Could you check a few things on this model? Use its own coordinates, in mm. Round coordinates to 2 decimals unless told otherwise and drop trailing zeros. Order: outer loops, then holes, each group sorted by start corner. A loop starts at its lowest first (then second) coordinate and runs counter-clockwise, first axis right, second up. Notation, with made-up numbers: (43.25, 69.25) -> (85.25, 69.25) arc R26 ccw to (85.25, 94.25) -> close; hole circle Ø4 at (-14, 16). An arc over 180 degrees is marked (long way). One line per question, with ' | ' between items.
```python
from build123d import *

# Parameters (mm, degrees)
SKETCH1_R           = 12.75
BOSS_EXTRUDE1_DEPTH = 12


with BuildPart() as part:
    # Sketch1 → Boss-Extrude1 (new body)
    with BuildSketch(Plane.XY):
        with BuildLine():
            Line((5, 0), (27, 0))
            ThreePointArc((27, 0), (30.535533906, 1.464466094), (32, 5))
            Line((32, 5), (32, 345))
            ThreePointArc((32, 345), (30.535533906, 348.535533906), (27, 350))
            Line((27, 350), (5, 350))
            ThreePointArc((5, 350), (1.464466094, 348.535533906), (0, 345))
            Line((0, 345), (0, 5))
            ThreePointArc((0, 5), (1.464466094, 1.464466094), (5, 0))
        make_face()
        with Locations((16, 20)):
            Circle(SKETCH1_R, mode=Mode.SUBTRACT)
    extrude(amount=BOSS_EXTRUDE1_DEPTH)


solid = part.part
```
1. If we mould it in two halves opening along Y, with no side actions, what happens to faces 1 (the face through (16, 350, 6)), 2 (the face through (32, 173, 6)), 3 (the face through (28.16, 23.83, 5.92))? For each: pulls with the +Y half, pulls with the -Y half, needs draft (parallel to the pull), parting line crosses it, or undercut.
From the geometry:
face 1: pulls with the +Y half | face 2: needs draft | face 3: undercut
2. I want a section at A-A on y = 20. List the corners of the cut face in (x, z) for me.
From the geometry:
outline: (0, 0) -> (3.25, 0) -> (3.25, 12) -> (0, 12) -> close; (28.75, 0) -> (32, 0) -> (32, 12) -> (28.75, 12) -> close
3. I want a section at C-C on z = 9.5. List the corners of the cut face in (x, y) for me, and give its area (3 significant figures).
From the geometry:
outline: (0, 5) arc R5 ccw to (5, 0) -> (27, 0) arc R5 ccw to (32, 5) -> (32, 345) arc R5 ccw to (27, 350) -> (5, 350) arc R5 ccw to (0, 345) -> close; hole circle Ø25.5 at (16, 20) | area: 10,700 mm²
4. I need wall thicknesses on probe 1 along Y at (x, z) = (16, 4); probe 2 along Y at (x, z) = (12, 1.25); probe 3 along Y at (x, z) = (1, 6.5). Which ranges of each line are inside material? Lowest first, please.
From the geometry:
probe 1: y = 0 to 7.25, 32.75 to 350 | probe 2: y = 0 to 7.89, 32.11 to 350 | probe 3: y = 2 to 348
5. I want a section at B-B on x = 14. List the corners of the cut face in (y, z) for me.
From the geometry:
outline: (0, 0) -> (7.41, 0) -> (7.41, 12) -> (0, 12) -> close; (32.59, 0) -> (350, 0) -> (350, 12) -> (32.59, 12) -> close
